The listing builds one solid part. Answer for the finished solid, in the listing's coordinates (mm). A direction names the side the tool comes from. Coordinates: 2 decimals unless noted, no trailing zeros. Order: outer loops, then holes, each group sorted by start corner. A loop starts at its lowest first (then second) coordinate and runs counter-clockwise, first axis right, second up. Notation, with made-up numbers: (-1, 25.25) - (5, 25.25) arc R29 ccw to (5, 56.25) - close; hole circle Ø2 at (34.5, -14). An arc over 180 degrees is marked (long way). One line per item, written item: value. Start each with the question number.
```python
from build123d import *

# Parameters (mm, degrees)
EXTRUDE_1_DEPTH = 6
CHAMFER_1_SIZE  = 2
CHAMFER_2_SIZE  = 2
CHAMFER_3_SIZE  = 2


with BuildPart() as part:
    # 草图1 → 凸台-拉伸1 (new, symmetric)
    with BuildSketch(Plane.XY):
        Polygon((0, 0), (0, 115), (12, 115), (12, 12), (46, 12), (46, 0), align=None)
    extrude(amount=EXTRUDE_1_DEPTH, both=True)

    # 倒角1
    chamfer_1_edges = [part.edges().sort_by_distance(p)[0] for p in [
        (12, 12, 0),
    ]]
    chamfer(chamfer_1_edges, length=CHAMFER_1_SIZE)

    # 倒角2
    chamfer_2_edges = [part.edges().sort_by_distance(p)[0] for p in [
        (0, 0, 0),
    ]]
    chamfer(chamfer_2_edges, length=CHAMFER_2_SIZE)

    # 倒角3
    chamfer_3_edges = [part.edges().sort_by_distance(p)[0] for p in [
        (12, 115, 0),
        (46, 12, 0),
    ]]
    chamfer(chamfer_3_edges, length=CHAMFER_3_SIZE)


solid = part.part
```
(1) The part is cut by section B-B on x = 23.5. Determine the outline of the cut face in (y, z).
(2) Consider probe 1 along X at (y, z) = (48.5, 0.25); probe 2 along X at (y, z) = (12.5, -4). Determine where each line is inside the solid, lowest interval first.
(3) The part is cut by section A-A on z = -3. Determine the outline of the cut face in (x, y), plus the area to 3 significant figures.
(4) Flat-ended cylindrical pins translate along their axes: pin 1 Ø3 at (y, z) = (24, -1.5) entering from +X; pin 2 Ø5 at (x, z) = (11, 4) entering from +Y; pin 3 Ø8 at (x, y) = (19, 56.5) entering from -Z; pin 4 Ø3.5 at (x, z) = (24.5, -2.5) entering from +Y. Find the tip coordinate at first contact, or state that the pin passes through.
(5) For faces 1 (the face through (29, 12, 0)), 2 (the face through (46, 5, 0)), determine the directions among +Z, -Z, +X, -X, +Y, -Y from which every point of the face is accessible in a straight line to the end or side of a thin tool.
Completed:
1. outline: (0, -6) - (12, -6) - (12, 6) - (0, 6) - close
2. probe 1: x = 0 to 12
2. probe 2: x = 0 to 13.5
3. outline: (0, 2) - (2, 0) - (46, 0) - (46, 10) - (44, 12) - (14, 12) - (12, 14) - (12, 113) - (10, 115) - (0, 115) - close
3. area: 1,780 mm2
4. pin 1: stops at x = 12
4. pin 2: stops at y = 115
4. pin 3: passes through
4. pin 4: stops at y = 12
5. face 1: +Z, -Z, +X, +Y
5. face 2: +Z, -Z, +X, +Y, -Y
